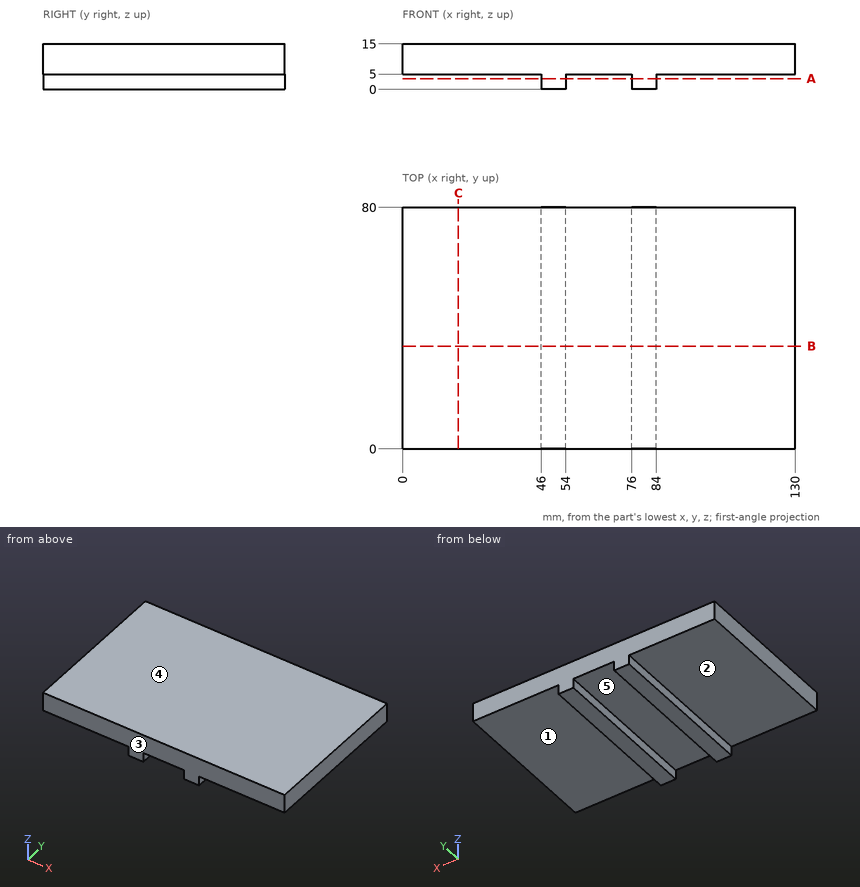
Here's the drawing with two shaded views (mm, measured from the low corner). I have some questions. A direction names the side the tool comes from. Coordinates: 2 decimals unless noted, no trailing zeros. Order: outer loops, then holes, each group sorted by start corner. A loop starts at its lowest first (then second) coordinate and runs counter-clockwise, first axis right, second up. Notation, with made-up numbers: M -28.75,-32 L -5.75,-32 A18 ccw -5.75,-22 Z; hole C -33,-39 d5. An arc over 180 degrees is marked long. Write item = value, one per line.
(1) For pin 1 Ø2 at (y, z) = (46, 3) entering from +X; pin 2 Ø17.5 at (x, y) = (67, 40) entering from -Z; pin 3 Ø2.5 at (y, z) = (36.5, 1.5) entering from -X, each with a flat end and sliding along its axis, tell me the tip position at first contact or that it passes through.
Results are:
pin_1 = 84
pin_2 = 5
pin_3 = 46
(2) Suppose I cut it at C-C on x = 18.5. Please give me the cut outline in (y, z).
Results are:
outline = M 0,5 L 80,5 L 80,15 L 0,15 Z
(3) If we mould it in two halves opening along X, with no side actions, what happens to the marked faces 4 and 5? For each: pulls with the +X half, pulls with the -X half, needs draft (parallel to the pull), parting line crosses it, or undercut.
Results are:
face_4 = needs draft
face_5 = undercut
(4) I need wall thicknesses on line 1 along X through (y, z) = (66, 3.5); line 2 along Z through (x, y) = (117, 7). Which ranges of each line are inside material? Lowest first, please. Write a range as [from, to].
Results are:
line_1 = [46, 54], [76, 84]
line_2 = [5, 15]
(5) Suppose I cut it at B-B on y = 34. Please give me the cut outline in (x, z).
Results are:
outline = M 0,5 L 46,5 L 46,0 L 54,0 L 54,5 L 76,5 L 76,0 L 84,0 L 84,5 L 130,5 L 130,15 L 0,15 Z
(6) For the marked faces 1, 2 and 3, which set-ups out of +Z, -Z, +X, -X, +Y, -Y let a thin tool reach every point of the face, with its end or its side?
Results are:
face_1 = -Z, +X, +Y, -Y
face_2 = -Z, -X, +Y, -Y
face_3 = +Z, -Z, +X, -X, -Y
(7) Suppose I cut it at A-A on z = 3.5. Please give me the cut outline in (x, y).
Results are:
outline = M 46,0 L 54,0 L 54,80 L 46,80 Z; M 76,0 L 84,0 L 84,80 L 76,80 Z
